```python
from build123d import *

# Parameters (mm, degrees)
SKETCH_1_W                = 160
SKETCH_1_H                = 300
EXTRUDE_1_DEPTH           = 12
CUT_EXTRUDE_1_DEPTH       = 171.423003142
HOLE_WIZARD_3_D           = 3.2
HOLE_WIZARD_3_CBORE_D     = 6
HOLE_WIZARD_3_CBORE_DEPTH = 7
HOLE_WIZARD_M5_1_D        = 4.2
CHAMFER_1_SIZE            = 5
SKETCH_29_W               = 70
SKETCH_29_H               = 45
SKETCH_29_W_2             = 75
CUT_EXTRUDE_3_DEPTH       = 171.423003142
FILLET_1_R                = 5
HOLE_WIZARD_M6_1_D        = 5


with BuildPart() as part:
    # 草图1 → 凸台-拉伸1 (new body)
    with BuildSketch(Plane(origin=(0, 0, 0), x_dir=(1, 0, 0), z_dir=(0, 1, 0))):
        Rectangle(SKETCH_1_W, SKETCH_1_H)
    extrude(amount=EXTRUDE_1_DEPTH)

    # 草图6 → 切除-拉伸1 (cut, through all)
    with BuildSketch(Plane(origin=(0, 12, 0), x_dir=(1, 0, 0), z_dir=(0, 1, 0))):
        with BuildLine():
            Line((-20, -74), (20, -74))
            ThreePointArc((20, -74), (30, -84), (20, -94))
            Line((20, -94), (-20, -94))
            ThreePointArc((-20, -94), (-30, -84), (-20, -74))
        make_face()
    extrude(amount=-CUT_EXTRUDE_1_DEPTH, mode=Mode.SUBTRACT)

    # Hole Wizard 3 (through all)
    with Locations(Plane(origin=(0, 0, 0), x_dir=(-1, 0, 0), z_dir=(0, -1, 0))):
        with Locations((35, 114), (-35, 114), (45, -56.5), (-45, -56.5)):
            CounterBoreHole(HOLE_WIZARD_3_D / 2, HOLE_WIZARD_3_CBORE_D / 2, HOLE_WIZARD_3_CBORE_DEPTH)

    # M5 螺纹孔1 (through all)
    with Locations(Plane(origin=(0, 12, 0), x_dir=(1, 0, 0), z_dir=(0, 1, 0))):
        with Locations((-57, -109), (57, -109)):
            Hole(HOLE_WIZARD_M5_1_D / 2)

    # 倒角1
    chamfer_1_edges = [part.edges().sort_by_distance(p)[0] for p in [
        (80, 6, 150),
        (-80, 6, 150),
        (-80, 6, -150),
        (80, 6, -150),
    ]]
    chamfer(chamfer_1_edges, length=CHAMFER_1_SIZE)

    # 草图29 → 切除-拉伸3 (cut, through all)
    with BuildSketch(Plane(origin=(0, 12, 0), x_dir=(1, 0, 0), z_dir=(0, 1, 0))):
        with Locations((10, 53.5)):
            Rectangle(SKETCH_29_W, SKETCH_29_H)
        with Locations((-6.5, -12)):
            Rectangle(SKETCH_29_W_2, SKETCH_29_H)
    extrude(amount=-CUT_EXTRUDE_3_DEPTH, mode=Mode.SUBTRACT)

    # 圆角1
    fillet_1_edges = [part.edges().sort_by_distance(p)[0] for p in [
        (31, 6, -10.5),
        (31, 6, 34.5),
        (-44, 6, 34.5),
        (-44, 6, -10.5),
        (45, 6, -76),
        (45, 6, -31),
        (-25, 6, -31),
        (-25, 6, -76),
    ]]
    fillet(fillet_1_edges, radius=FILLET_1_R)

    # M6 螺纹孔1 (through all)
    with Locations(Plane(origin=(0, 12, 0), x_dir=(1, 0, 0), z_dir=(0, 1, 0))):
        with Locations((-54, 93), (29, 93), (-54, 23), (29, 23)):
            Hole(HOLE_WIZARD_M6_1_D / 2)


solid = part.part
```
Work out the finished part from the listing and answer in its coordinate system (mm). A direction names the side the tool comes from. Round coordinates to 2 decimals unless told otherwise and drop trailing zeros.
(1) The mould has two halves that part along X. Classify faces 4 (the flat face through (80, 6, 2)), 5 (the flat face through (0, 6, 94)), 6 (the flat face through (-1, 6, 150)), 7 (the flat face through (-80, 6, 2)): pulls with the +X half, pulls with the -X half, needs draft (parallel to the pull), parting line crosses it, or undercut.
Computed values:
face 4: pulls with the +X half
face 5: undercut
face 6: needs draft
face 7: pulls with the -X half
(2) Each of these flat-tipped pins is pushed along its axis until it touches: P1, Ø3, axis at x = 29, z = -93, coming from the +Y side; P2, Ø8, axis at x = 45, z = 56.5, coming from the -Y side; P3, Ø5, axis at x = 35, z = -114, coming from the -Y side. Where does it stop, or does it pass through?
Computed values:
P1: passes through
P2: stops at y = 0
P3: stops at y = 7
(3) The part is cut by section A-A, the plane y = 3. Give the number of separate pieces and of enclosed holes in the cut face, and give its area (3 significant figures).
Computed values:
separate pieces: 1
enclosed holes: 13
area: 40,100 mm2
(4) Find the intervals of material crossed by L1, parallel to Z at x = -54, y = 3.25; L2, parallel to Z at x = 5, y = 1; L3, parallel to Z at x = -35, y = 5.25, in increasing order.
Computed values:
L1: z = -150 to -95.5, -90.5 to -25.5, -20.5 to 150
L2: z = -150 to -76, -31 to -10.5, 34.5 to 74, 94 to 150
L3: z = -150 to -117, -111 to -10.5, 34.5 to 150
(5) For faces 1 (the cylindrical face through (30, 6, 84)), 2 (the flat face through (-46, 7, 58)), 3 (the flat face through (-1, 6, -150)), determine the directions among +Z, -Z, +X, -X, +Y, -Y from which every point of the face is accessible in a straight line to the end or side of a thin tool.
Computed values:
face 1: +Y, -Y
face 2: -Y
face 3: -Z, +X, -X, +Y, -Y
